```python
from build123d import *

# Parameters (mm, degrees)
BOSS_EXTRUDE1_DEPTH = 10
SKETCH3_R           = 1
BOSS_EXTRUDE2_DEPTH = 1
SKETCH4_R           = 1
CUT_EXTRUDE1_DEPTH  = 1


with BuildPart() as part:
    # Sketch1 → Boss-Extrude1 (new, symmetric)
    with BuildSketch(Plane.XY):
        with BuildLine():
            Line((-17.5, -17.5), (17.5, -17.5))
            ThreePointArc((17.5, -17.5), (21.035533906, -16.035533906), (22.5, -12.5))
            Line((22.5, -12.5), (22.5, 12.5))
            ThreePointArc((22.5, 12.5), (21.035533906, 16.035533906), (17.5, 17.5))
            Line((17.5, 17.5), (-17.5, 17.5))
            ThreePointArc((-17.5, 17.5), (-21.035533906, 16.035533906), (-22.5, 12.5))
            Line((-22.5, 12.5), (-22.5, -12.5))
            ThreePointArc((-22.5, -12.5), (-21.035533906, -16.035533906), (-17.5, -17.5))
        make_face()
    extrude(amount=BOSS_EXTRUDE1_DEPTH, both=True)

    # Sketch3 → Boss-Extrude2 (add)
    # profile 1 of 3: a face of its own
    with BuildSketch(Plane(origin=(0, 0, -3), x_dir=(-1, 0, 0), z_dir=(0, 0, -1))):
        with BuildLine():
            Line((-8, 17.5), (-12, 17.5))
            Line((-12, 17.5), (-12, 26.5))
            ThreePointArc((-12, 26.5), (-11.707106781, 27.207106781), (-11, 27.5))
            Line((-11, 27.5), (-9, 27.5))
            ThreePointArc((-9, 27.5), (-8.292893219, 27.207106781), (-8, 26.5))
            Line((-8, 26.5), (-8, 17.5))
        make_face()
    # profile 2 of 3: a face of its own
    with BuildSketch(Plane(origin=(0, 0, -3), x_dir=(-1, 0, 0), z_dir=(0, 0, -1))):
        with BuildLine():
            Line((8, 17.5), (12, 17.5))
            Line((12, 17.5), (12, 26.5))
            ThreePointArc((12, 26.5), (11.707106781, 27.207106781), (11, 27.5))
            Line((11, 27.5), (9, 27.5))
            ThreePointArc((9, 27.5), (8.292893219, 27.207106781), (8, 26.5))
            Line((8, 26.5), (8, 17.5))
        make_face()
    # profile 3 of 3: a face of its own
    with BuildSketch(Plane(origin=(0, 0, -3), x_dir=(-1, 0, 0), z_dir=(0, 0, -1))):
        with BuildLine():
            Line((-2.5, -17.5), (2.5, -17.5))
            Line((2.5, -17.5), (2.5, -26.5))
            ThreePointArc((2.5, -26.5), (2.207106781, -27.207106781), (1.5, -27.5))
            Line((1.5, -27.5), (-1.5, -27.5))
            ThreePointArc((-1.5, -27.5), (-2.207106781, -27.207106781), (-2.5, -26.5))
            Line((-2.5, -26.5), (-2.5, -17.5))
        make_face()
        with Locations((0, -22.5)):
            Circle(SKETCH3_R, mode=Mode.SUBTRACT)
    extrude(amount=-BOSS_EXTRUDE2_DEPTH)

    # Sketch4 → Cut-Extrude1 (cut)
    with BuildSketch(Plane(origin=(0, 0, -3), x_dir=(-1, 0, 0), z_dir=(0, 0, -1))):
        with Locations((-10, 22.5)):
            Circle(SKETCH4_R)
        with Locations((10, 22.5)):
            Circle(SKETCH4_R)
    extrude(amount=-CUT_EXTRUDE1_DEPTH, mode=Mode.SUBTRACT)


solid = part.part
```
For this review, take the finished solid that the model builds, in its own axes (mm). A direction names the side the tool comes from. Coordinates: 2 decimals unless noted, no trailing zeros. Write each loop counter-clockwise with the first axis right and the second up, starting at its lowest first coordinate (ties: lowest second). Pieces come first, ordered by that corner, then holes. Notation, with made-up numbers: (52.25, 69) - (70.25, 69) arc R27 ccw to (70.25, 105) - close; hole circle Ø6 at (50.5, 21.5). An arc over 180 degrees is marked (long way). Put each result on its own line as item: value.
1. Wall thickness on probe 1 along Y at (x, z) = (0, -2.25); probe 2 along Y at (x, z) = (10, -2.55); probe 3 along Y at (x, z) = (14, 4): over which ranges is each line inside the solid? List them lowest first.
Values found:
probe 1: -27.5 to -23.5, -21.5 to 17.5
probe 2: -17.5 to 21.5, 23.5 to 27.5
probe 3: -17.5 to 17.5
2. Add section C-C, the plane y = -22.5. Give the boundary of the cut face in (x, z), then the cut area to 3 significant figures.
Values found:
outline: (-2.5, -3) - (-1, -3) - (-1, -2) - (-2.5, -2) - close; (1, -3) - (2.5, -3) - (2.5, -2) - (1, -2) - close
area: 3.00 mm²
3. Add section D-D, the plane z = -8.25. Give the boundary of the cut face in (x, y), then the cut area to 3 significant figures.
Values found:
outline: (-22.5, -12.5) arc R5 ccw to (-17.5, -17.5) - (17.5, -17.5) arc R5 ccw to (22.5, -12.5) - (22.5, 12.5) arc R5 ccw to (17.5, 17.5) - (-17.5, 17.5) arc R5 ccw to (-22.5, 12.5) - close
area: 1,550 mm²
4. For pin 1 (5.5 mm diameter, centred on x = 0, y = -24.5, fed in from +Z); pin 2 (2.5 mm diameter, centred on x = 0, y = -21, fed in from -Z); pin 3 (1 mm diameter, centred on x = 13, z = 4, fed in from +Y), all flat-tipped, find the tip position at first contact; note any pin that passes through.
Values found:
pin 1: z = -2
pin 2: z = -3
pin 3: y = 17.5
5. Machinability: for faces 4 (the flat face through (0, -21, -2)), 5 (the flat face through (10, 21, -3)), 6 (the flat face through (0, -21, -3)), which of the approach directions +Z, -Z, +X, -X, +Y, -Y give a long, thin tool a straight path to every point of the face, cutting with its end or side? Answer none if there is none.
Values found:
face 4: +Z, +X, -X, -Y
face 5: -Z, +X, -X, +Y
face 6: -Z, +X, -X, -Y
6. Mouldability with a two-part tool opening along Y and no side actions: class faces 1 (the cylindrical face through (-21.07, -16, 0.14)), 2 (the flat face through (-10, 21, -2)), 3 (the cylindrical face through (0.217, -23.476, -2.507)) as released by +Y, released by -Y, zero draft, split by the parting line, or undercut.
Values found:
face 1: released by -Y
face 2: zero draft
face 3: undercut
7. Add section A-A, the plane y = 22.5. Give the boundary of the cut face in (x, z), then the cut area to 3 significant figures.
Values found:
outline: (-12, -3) - (-11, -3) - (-11, -2) - (-12, -2) - close; (-9, -3) - (-8, -3) - (-8, -2) - (-9, -2) - close; (8, -3) - (9, -3) - (9, -2) - (8, -2) - close; (11, -3) - (12, -3) - (12, -2) - (11, -2) - close
area: 4.00 mm²
8. Add section B-B, the plane x = -10. Give the boundary of the cut face in (y, z), then the cut area to 3 significant figures.
Values found:
outline: (-17.5, -10) - (17.5, -10) - (17.5, -3) - (21.5, -3) - (21.5, -2) - (17.5, -2) - (17.5, 10) - (-17.5, 10) - close; (23.5, -3) - (27.5, -3) - (27.5, -2) - (23.5, -2) - close
area: 708 mm²
